Source: three-view drawing plus pictorial views. Frame: mm from the lowest corner of the part. Give positions to 0.01 mm unless a question says otherwise; leave off trailing zeros. Write each loop counter-clockwise with the first axis right and the second up, starting at its lowest first coordinate (ties: lowest second). Pieces come first, ordered by that corner, then holes.
Q1. Pin query (flat end, axial travel): pin 1 (10 mm diameter, centred on x = 37.5, z = 89.5, fed in from -Y); pin 2 (18 mm diameter, centred on y = 39, z = 49, fed in from +X); pin 3 (10.5 mm diameter, centred on x = 28.5, z = 59, fed in from +Y). Return the tip coordinate at first contact, or that it passes through.
Q2. Cut plane D-D on z = 34. Return the cut outline in (x, y), plus the area to 3 significant figures.
Q3. Cut plane C-C on y = 30. Return the cut outline in (x, z), plus the area to 3 significant figures.
Q4. Line query: L1, parallel to X at y = 45.5, z = 57.5; L2, parallel to Y at x = 36, z = 14; L3, parallel to Y at x = 30.5, z = 88. Output: solid intervals per line, ascending.
Q5. Cut plane B-B on x = 15.5. Return the cut outline in (y, z), plus the area to 3 significant figures.
Q6. Draft query along X for the marked faces 1, 2, 3 and 4. Return one class per face: pulls with the +X half, pulls with the -X half, needs draft (parallel to the pull), parting line crosses it, or undercut.
Q7. Cut plane A-A on z = 91.5. Return the cut outline in (x, y).
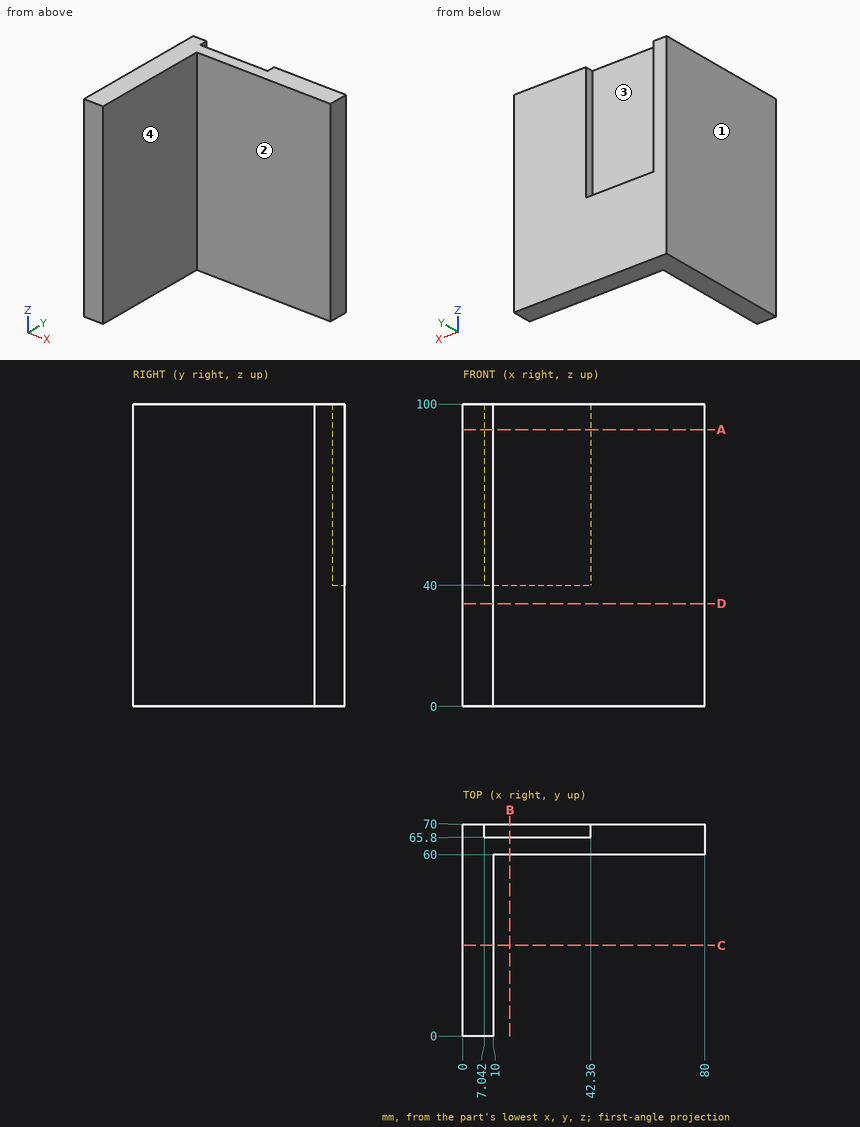
Data:
1. pin 1: stops at y = 60
1. pin 2: stops at x = 10
1. pin 3: stops at y = 65.8
2. outline: (0, 0) - (10, 0) - (10, 60) - (80, 60) - (80, 70) - (0, 70) - close
2. area: 1,400 mm2
3. outline: (0, 0) - (10, 0) - (10, 100) - (0, 100) - close
3. area: 1,000 mm2
4. L1: x = 0 to 10
4. L2: y = 60 to 70
4. L3: y = 60 to 65.8
5. outline: (60, 0) - (70, 0) - (70, 40) - (65.8, 40) - (65.8, 100) - (60, 100) - close
5. area: 748 mm2
6. face 1: pulls with the -X half
6. face 2: needs draft
6. face 3: undercut
6. face 4: pulls with the +X half
7. outline: (0, 0) - (10, 0) - (10, 60) - (80, 60) - (80, 70) - (42.36, 70) - (42.36, 65.8) - (7.04, 65.8) - (7.04, 70) - (0, 70) - close
